from build123d import *

# Parameters (mm, degrees)
BACK_PLATE_DEPTH            = 10
BASE_PLATE_DEPTH            = 10
BEARING_BLOCK_DEPTH         = 30
BACK_PLATE_HOLES_SKETCH_R   = 4
BACK_PLATE_HOLES_2X_8_DEPTH = 10
BASE_PLATE_HOLES_SKETCH_R   = 4
BASE_PLATE_HOLES_2X_8_DEPTH = 10


with BuildPart() as part:
    # Back Plate Sketch → Back Plate (new body)
    with BuildSketch(Plane.XY):
        with BuildLine():
            Line((0, 0), (80, 0))
            Line((80, 0), (80, 35))
            ThreePointArc((80, 35), (78.535533906, 38.535533906), (75, 40))
            Line((75, 40), (5, 40))
            ThreePointArc((5, 40), (1.464466094, 38.535533906), (0, 35))
            Line((0, 35), (0, 0))
        make_face()
    extrude(amount=BACK_PLATE_DEPTH)

    # Base Plate Sketch → Base Plate (add)
    with BuildSketch(Plane.XZ):
        with BuildLine():
            Line((0, 10), (0, 35))
            ThreePointArc((0, 35), (1.464466094, 38.535533906), (5, 40))
            Line((5, 40), (20, 40))
            Line((20, 40), (20, 10))
            Line((20, 10), (0, 10))
        make_face()
        with BuildLine():
            Line((80, 10), (80, 35))
            ThreePointArc((80, 35), (78.535533906, 38.535533906), (75, 40))
            Line((75, 40), (60, 40))
            Line((60, 40), (60, 10))
            Line((60, 10), (80, 10))
        make_face()
    extrude(amount=-BASE_PLATE_DEPTH)

    # Bearing Block Sketch → Bearing Block (add)
    with BuildSketch(Plane.XZ):
        with BuildLine():
            Line((20, 10), (20, 40))
            Line((20, 40), (24.655964266, 40))
            ThreePointArc((24.655964266, 40), (39.655964266, 25), (54.655964266, 40))
            Line((54.655964266, 40), (60, 40))
            Line((60, 40), (60, 10))
            Line((60, 10), (20, 10))
        make_face()
    extrude(amount=-BEARING_BLOCK_DEPTH)

    # Back Plate Holes Sketch → Back Plate Holes 2xØ8 (cut)
    with BuildSketch(Plane.XY.offset(10)):
        with Locations((10, 30)):
            Circle(BACK_PLATE_HOLES_SKETCH_R)
        with Locations((70.447162461, 30)):
            Circle(BACK_PLATE_HOLES_SKETCH_R)
    extrude(amount=-BACK_PLATE_HOLES_2X_8_DEPTH, mode=Mode.SUBTRACT)

    # Base Plate Holes Sketch → Base Plate Holes 2xØ8 (cut)
    with BuildSketch(Plane(origin=(0, 10, 0), x_dir=(1, 0, 0), z_dir=(0, 1, 0))):
        with Locations(Location((10, -30, 0), (0, 0, 270))):
            Circle(BASE_PLATE_HOLES_SKETCH_R)
        with Locations(Location((70.017117794, -30, 0), (0, 0, 270))):
            Circle(BASE_PLATE_HOLES_SKETCH_R)
    extrude(amount=-BASE_PLATE_HOLES_2X_8_DEPTH, mode=Mode.SUBTRACT)


solid = part.part
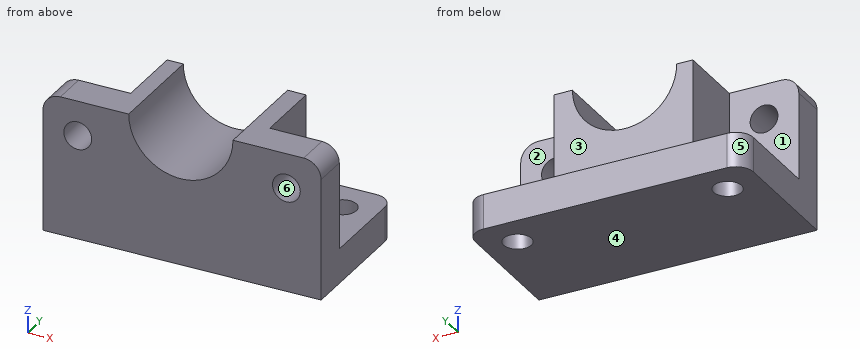
Work out the finished part from the listing and answer in its coordinate system (mm). Face numbers are marked on the shaded views. A direction names the side the tool comes from. Coordinates: 2 decimals unless noted, no trailing zeros. Write each loop counter-clockwise with the first axis right and the second up, starting at its lowest first coordinate (ties: lowest second). Pieces come first, ordered by that corner, then holes. Notation, with made-up numbers: (77, -21) - (97, -21) arc R15 cw to (97, -3) - close; hole circle Ø4 at (44.5, 63.5). An arc over 180 degrees is marked (long way). One line per question, with ' | ' between items.
1) Find section D-D, the plane y = 16. Determine the outline of the cut face in (x, z), and give its area (3 significant figures).
Checks:
outline: (0, 0) - (80, 0) - (80, 10) - (60, 10) - (60, 40) - (54.66, 40) arc R15 cw to (24.66, 40) - (20, 40) - (20, 10) - (0, 10) - close | area: 1,650 mm2
2) Find section C-C, the plane y = 31.5. Determine the outline of the cut face in (x, z), and give its area (3 significant figures).
Checks:
outline: (0, 0) - (6.29, 0) - (6.29, 10) - (0, 10) - close; (13.71, 0) - (66.74, 0) - (66.74, 10) - (13.71, 10) - close; (74.16, 0) - (80, 0) - (80, 10) - (74.16, 10) - close | area: 652 mm2
3) For the marked faces 1, 2 and 3, determine the directions among +Z, -Z, +X, -X, +Y, -Y from which every point of the face is accessible in a straight line to the end or side of a thin tool.
Checks:
face 1: +Z, -X, +Y | face 2: +Z, +X, +Y | face 3: +Z, +X, -X, +Y
4) Flat-ended cylindrical pins translate along their axes: P1, Ø22, axis at x = 7, z = 22.5, coming from the +Y side; P2, Ø12, axis at x = 18.5, z = 35.5, coming from the +Y side; P3, Ø5, axis at y = 19.5, z = 16.5, coming from the +X side. Find the tip coordinate at first contact, or state that the pin passes through.
Checks:
P1: y = 10 | P2: y = 30 | P3: x = 60
5) Consider probe 1 along Y at (x, z) = (10, 2); probe 2 along Y at (x, z) = (44, 25.5); probe 3 along Y at (x, z) = (62.5, 12.5). Determine where each line is inside the solid, lowest interval first. Write a range as [from, to].
Checks:
probe 1: [0, 26], [34, 40] | probe 2: [0, 30] | probe 3: [0, 10]
6) Find section A-A, the plane x = 10. Determine the outline of the cut face in (y, z), and give its area (3 significant figures).
Checks:
outline: (0, 0) - (26, 0) - (26, 10) - (10, 10) - (10, 26) - (0, 26) - close; (0, 34) - (10, 34) - (10, 40) - (0, 40) - close; (34, 0) - (40, 0) - (40, 10) - (34, 10) - close | area: 540 mm2
7) Find section B-B, the plane z = 5. Determine the outline of the cut face in (x, y), and give its area (3 significant figures).
Checks:
outline: (0, 0) - (80, 0) - (80, 35) arc R5 ccw to (75, 40) - (5, 40) arc R5 ccw to (0, 35) - close; hole circle Ø8 at (10, 30); hole circle Ø8 at (70.45, 30) | area: 3,090 mm2
8) The mould has two halves that part along Z. Classify the marked faces 4, 5 and 6: +Z half, -Z half, draft (parallel to the pull), parting line (faces both ways), or undercut.
Checks:
face 4: -Z half | face 5: draft | face 6: undercut
